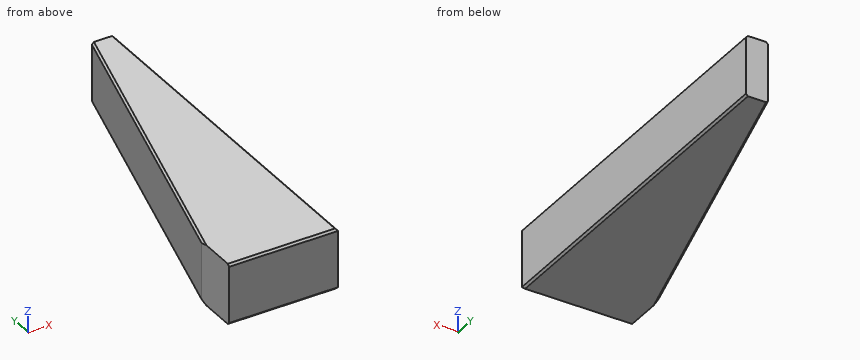
```python
from build123d import *

# Parameters (mm, degrees)
EXTRUDE_1_DEPTH     = 15
CHAMFER_1_SIZE      = 0.5
SKETCH_7_W          = 5.5
SKETCH_7_H          = 20.166666667
SKETCH_7_W_2        = 3
SKETCH_7_H_2        = 20
CUT_EXTRUDE_1_DEPTH = 116


with BuildPart() as part:
    # 草图1 → 凸台-拉伸1 (new body)
    with BuildSketch(Plane.XY):
        Polygon((0, 0), (30, 0), (30, 110), align=None)
    extrude(amount=EXTRUDE_1_DEPTH)

    # 倒角1
    chamfer_1_edges = [part.edges().sort_by_distance(p)[0] for p in [
        (30, 55, 15),
        (30, 55, 0),
        (15, 55, 15),
        (15, 0, 0),
        (15, 55, 0),
        (15, 0, 15),
    ]]
    chamfer(chamfer_1_edges, length=CHAMFER_1_SIZE)

    # 草图7 → 切除-拉伸1 (cut, through all)
    with BuildSketch(Plane.XY.offset(15)):
        with Locations((27.25, 99.916666666)):
            Rectangle(SKETCH_7_W, SKETCH_7_H)
        with Locations((1.5, 10)):
            Rectangle(SKETCH_7_W_2, SKETCH_7_H_2)
    extrude(amount=-CUT_EXTRUDE_1_DEPTH, mode=Mode.SUBTRACT)


solid = part.part
```
For this review, take the finished solid that the model builds, in its own axes (mm). Round coordinates to 2 decimals unless told otherwise and drop trailing zeros. Loops run counter-clockwise (first coordinate to the right, second up) from the corner with the lowest first, then second, coordinate; pieces in that order, holes last.
Q1. Insertion check: pin 1 Ø6 at (y, z) = (78.5, 2) entering from -X. The pin has a flat end and moves straight along its axis. Give the tip position at first contact, or say it passes through.
Result sheet:
pin 1: stops at x = 20.59
Q2. Add section A-A on z = 8.5. Write out the cut boundary in (x, y).
Result sheet:
outline: (3, 0) - (30, 0) - (30, 89.83) - (24.5, 89.83) - (3, 11) - close
Q3. Add section C-C on x = 11. Write out the cut boundary in (y, z), plus the area to 3 significant figures.
Result sheet:
outline: (0, 0.5) - (0.5, 0) - (38.43, 0) - (40.33, 0.5) - (40.33, 14.5) - (38.43, 15) - (0.5, 15) - (0, 14.5) - close
area: 604 mm2
Q4. To check wall thickness, follow line 1 along X through (y, z) = (84.5, 11.75); line 2 along X through (y, z) = (46.5, 2.5). State the ranges of each line that lie inside material, in increasing order.
Result sheet:
line 1: x = 23.05 to 30
line 2: x = 12.68 to 30
Q5. Add section B-B on y = 60. Write out the cut boundary in (x, z).
Result sheet:
outline: (16.36, 0.5) - (16.88, 0) - (29.5, 0) - (30, 0.5) - (30, 14.5) - (29.5, 15) - (16.88, 15) - (16.36, 14.5) - close
